Build history of the part. All positions in model axes, mm. Coordinates: 2 decimals unless noted, no trailing zeros. Order: outer loops, then holes, each group sorted by start corner. A loop starts at its lowest first (then second) coordinate and runs counter-clockwise, first axis right, second up. Notation, with made-up numbers: (84, 15.5) - (97, 15.5) arc R9 cw to (97, 30.5) - close; hole circle Ø5 at (12.5, 7). An arc over 180 degrees is marked (long way). Write each question's results on one line, items separated by ' | '. Start each with the question number.
from build123d import *

# Parameters (mm, degrees)
SKETCH1_W            = 20
SKETCH1_H            = 10
BOSS_EXTRUDE1_DEPTH  = 10
M5_TAPPED_HOLE1_D    = 4.2
M4_CLEARANCE_HOLE1_D = 4.5
CHAMFER1_SIZE        = 0.5


with BuildPart() as part:
    # Sketch1 → Boss-Extrude1 (new, symmetric)
    with BuildSketch(Plane(origin=(0, 0, 0), x_dir=(1, 0, 0), z_dir=(0, 1, 0))):
        Rectangle(SKETCH1_W, SKETCH1_H)
    extrude(amount=BOSS_EXTRUDE1_DEPTH, both=True)

    # M5 Tapped Hole1 (through all)
    with Locations(Plane.XY.offset(5)):
        with Locations((0, 5)):
            Hole(M5_TAPPED_HOLE1_D / 2)

    # M4 Clearance Hole1 (through all)
    with Locations(Plane(origin=(0, 10, 0), x_dir=(1, 0, 0), z_dir=(0, 1, 0))):
        with Locations((6.5, 0), (-6.5, 0)):
            Hole(M4_CLEARANCE_HOLE1_D / 2)

    # Chamfer1
    chamfer1_edges = [part.edges().sort_by_distance(p)[0] for p in [
        (-10, 10, 0),
        (10, 10, 0),
        (-10, -10, 0),
        (10, -10, 0),
    ]]
    chamfer(chamfer1_edges, length=CHAMFER1_SIZE)


solid = part.part
Item 1: Pull direction Y, two halves, no side cores. Call faces 1 (the flat face through (0, 0, 5)), 2 (the cylindrical face through (0.273, 7.082, -0.07)), 3 (the flat face through (0, 10, 0)), 4 (the flat face through (0, -10, 0)): released by +Y, released by -Y, zero draft, split by the parting line, or undercut.
Item 2: Slice it at B-B (y = 5). Write the cut outline in (x, z), then the cut area to 3 significant figures.
Item 3: Slice it at C-C (x = 6.5). Write the cut outline in (y, z), then the cut area to 3 significant figures.
Item 4: Slice it at A-A (z = 0). Write the cut outline in (x, y), then the cut area to 3 significant figures.
Item 5: Slice it at D-D (z = 3). Write the cut outline in (x, y).
Item 6: Probe probe 1 along Z at (x, y) = (6.5, -3.75); probe 2 along Y at (x, z) = (0, -1.5); probe 3 along X at (y, z) = (1.5, -0.25). List the from-to ranges inside material, lowest first.
Item 7: Flat gauge pin, fed straight in: P1, Ø2.5, axis at x = 6.5, z = 0, coming from the +Y side. Where does the tip first touch, or does it go through?
Resolved:
1) face 1: zero draft | face 2: undercut | face 3: released by +Y | face 4: released by -Y
2) outline: (-10, -5) - (-2.1, -5) - (-2.1, 5) - (-10, 5) - close; (2.1, -5) - (10, -5) - (10, 5) - (2.1, 5) - close; hole circle Ø4.5 at (-6.5, 0); hole circle Ø4.5 at (6.5, 0) | area: 126 mm^2
3) outline: (-10, -5) - (10, -5) - (10, -2.25) - (-10, -2.25) - close; (-10, 2.25) - (10, 2.25) - (10, 5) - (-10, 5) - close | area: 110 mm^2
4) outline: (-10, -9.5) - (-9.5, -10) - (-8.75, -10) - (-8.75, 10) - (-9.5, 10) - (-10, 9.5) - close; (-4.25, -10) - (4.25, -10) - (4.25, 10) - (-4.25, 10) - close; (8.75, -10) - (9.5, -10) - (10, -9.5) - (10, 9.5) - (9.5, 10) - (8.75, 10) - close; hole circle Ø4.2 at (0, 5) | area: 206 mm^2
5) outline: (-10, -9.5) - (-9.5, -10) - (9.5, -10) - (10, -9.5) - (10, 9.5) - (9.5, 10) - (-9.5, 10) - (-10, 9.5) - close; hole circle Ø4.2 at (0, 5)
6) probe 1: -5 to -2.25, 2.25 to 5 | probe 2: -10 to 2.9, 7.1 to 10 | probe 3: -10 to -8.74, -4.26 to 4.26, 8.74 to 10
7) P1: through
